Build history of the part. All positions in model axes, mm. A direction names the side the tool comes from. Coordinates: 2 decimals unless noted, no trailing zeros. Write each loop counter-clockwise with the first axis right and the second up, starting at its lowest first coordinate (ties: lowest second). Pieces come first, ordered by that corner, then holes. Notation, with made-up numbers: (-21.75, -18.75) -> (26.25, -18.75) arc R18 ccw to (26.25, 1.25) -> close; hole circle Ø7 at (58.25, 40). An arc over 180 degrees is marked (long way). Write each question's results on one line, items separated by ' | '. Start each with the question number.
Q1. Tool access for faces 5 (the face through (2, -8.75, 0)), 6 (the face through (5.4, -6.24, 0.01)), 7 (the face through (4, -3.75, 0)), 8 (the face through (-5.2, 6.5, 0)): list every direction of +Z, -Z, +X, -X, +Y, -Y with a clear straight run to the whole face (end or side of a thin tool).
Q2. Two-plate mould, pull along X, no slides. Class faces 1 (the face through (0, -2, 0.65)), 2 (the face through (-5.72, 7.67, 0.01)), 3 (the face through (5.8, -6, 0)), 4 (the face through (2.377, -7.359, 0.009)): released by +X, released by -X, zero draft, split by the parting line, or undercut.
Q3. Saw through at A-A on y = -5.25. Give the cut face in (x, z), and give its area (3 significant figures).
Q4. Saw through at C-C on x = -1.2. Give the cut face in (y, z).
Q5. Saw through at B-B on z = -0.45. Give the cut face in (x, y), and give its area (3 significant figures).
Q6. Drop flat-ended pins along their axis: pin 1 Ø0.6 at (x, z) = (4.5, 0) entering from +Y; pin 2 Ø0.6 at (y, z) = (0.5, 0) entering from -X. Give the stop position or say it passes through.
Q7. Drill centre lines: line 1 (Y direction, x = 2.25, z = 0.2); line 2 (Y direction, x = -3.5, z = 0.1); line 3 (X direction, y = -4.5, z = -0.6). Where is each one in solid material? Low to high.
Q8. Saw through at D-D on x = 4. Give the cut face in (y, z), and give its area (3 significant figures).
from build123d import *

# Parameters (mm, degrees)
SKETCH1_W           = 11.6
SKETCH1_H           = 17.5
BOSS_EXTRUDE1_DEPTH = 0.65
SKETCH2_R           = 1.25
SKETCH2_R_2         = 0.5
CUT_EXTRUDE1_DEPTH  = 11.577925127
SKETCH3_W           = 3.6
SKETCH3_H           = 14.7
CUT_EXTRUDE2_DEPTH  = 11.577925127
SKETCH4_W           = 0.6
SKETCH4_H           = 1
CUT_EXTRUDE3_DEPTH  = 11.577925127
FILLET2_R           = 0.2
CUT_EXTRUDE4_DEPTH  = 11.577925127
FILLET3_R           = 1
CHAMFER1_SIZE       = 0.2
FILLET4_R           = 0.5


with BuildPart() as part:
    # Sketch1 → Boss-Extrude1 (new, symmetric)
    with BuildSketch(Plane.XY):
        Rectangle(SKETCH1_W, SKETCH1_H)
    extrude(amount=BOSS_EXTRUDE1_DEPTH, both=True)

    # Sketch2 → Cut-Extrude1 (cut, through all)
    with BuildSketch(Plane.XY.offset(0.65)):
        with Locations((1.8, -6.25)):
            Circle(SKETCH2_R)
        with Locations((-1.2, -6.25)):
            Circle(SKETCH2_R_2)
        with BuildLine():
            Line((4.7, -5.75), (4.9, -5.75))
            ThreePointArc((4.9, -5.75), (5.4, -6.25), (4.9, -6.75))
            Line((4.9, -6.75), (4.7, -6.75))
            ThreePointArc((4.7, -6.75), (4.2, -6.25), (4.7, -5.75))
        make_face()
    extrude(amount=-CUT_EXTRUDE1_DEPTH, mode=Mode.SUBTRACT)

    # Sketch3 → Cut-Extrude2 (cut, through all)
    with BuildSketch(Plane.XY.offset(0.65)):
        with Locations((-4, -1.4)):
            Rectangle(SKETCH3_W, SKETCH3_H)
        Polygon((5.8, -3.75), (1.8, -3.75), (-0.8, 8.75), (5.8, 8.75), align=None)
    extrude(amount=-CUT_EXTRUDE2_DEPTH, mode=Mode.SUBTRACT)

    # Sketch4 → Cut-Extrude3 (cut, through all)
    with BuildSketch(Plane.XY.offset(0.65)):
        with Locations((-5.5, 6.45)):
            Rectangle(SKETCH4_W, SKETCH4_H)
    extrude(amount=-CUT_EXTRUDE3_DEPTH, mode=Mode.SUBTRACT)

    # Fillet2
    fillet2_edges = [part.edges().sort_by_distance(p)[0] for p in [
        (-5.2, 5.95, 0),
    ]]
    fillet(fillet2_edges, radius=FILLET2_R)

    # Sketch5 → Cut-Extrude4 (cut, through all)
    with BuildSketch(Plane.XY.offset(0.65)):
        Polygon((-5.8, 7.05), (-5.576190754, 8.75), (-5.8, 8.75), align=None)
    extrude(amount=-CUT_EXTRUDE4_DEPTH, mode=Mode.SUBTRACT)

    # Fillet3
    fillet3_edges = [part.edges().sort_by_distance(p)[0] for p in [
        (-2.2, 5.95, 0),
        (1.8, -3.75, 0),
        (-0.8, 8.75, 0),
    ]]
    fillet(fillet3_edges, radius=FILLET3_R)

    # Chamfer1
    chamfer1_edges = [part.edges().sort_by_distance(p)[0] for p in [
        (-2.2, -8.75, 0),
        (5.8, -3.75, 0),
        (5.8, -8.75, 0),
    ]]
    chamfer(chamfer1_edges, length=CHAMFER1_SIZE)

    # Fillet4
    fillet4_edges = [part.edges().sort_by_distance(p)[0] for p in [
        (-5.576190754, 8.75, 0),
    ]]
    fillet(fillet4_edges, radius=FILLET4_R)


solid = part.part
Returned:
1) face 5: +Z, -Z, +X, -X, -Y | face 6: +Z, -Z | face 7: +Z, -Z, +X, +Y | face 8: +Z, -Z, -X, -Y
2) face 1: zero draft | face 2: released by -X | face 3: released by +X | face 4: undercut
3) outline: (-2.2, -0.65) -> (1.05, -0.65) -> (1.05, 0.65) -> (-2.2, 0.65) -> close; (2.55, -0.65) -> (5.8, -0.65) -> (5.8, 0.65) -> (2.55, 0.65) -> close | area: 8.45 mm2
4) outline: (-8.75, -0.65) -> (-6.75, -0.65) -> (-6.75, 0.65) -> (-8.75, 0.65) -> close; (-5.75, -0.65) -> (8.66, -0.65) -> (8.66, 0.65) -> (-5.75, 0.65) -> close
5) outline: (-5.8, 6.95) -> (-5.2, 6.95) -> (-5.2, 6.15) arc R0.2 ccw to (-5, 5.95) -> (-3.2, 5.95) arc R1 cw to (-2.2, 4.95) -> (-2.2, -8.55) -> (-2, -8.75) -> (5.6, -8.75) -> (5.8, -8.55) -> (5.8, -3.95) -> (5.6, -3.75) -> (2.61, -3.75) arc R1 cw to (1.63, -2.95) -> (-0.63, 7.95) arc R1 ccw to (-1.61, 8.75) -> (-5.14, 8.75) arc R0.5 ccw to (-5.63, 8.32) -> (-5.8, 7.05) -> close; hole circle Ø1 at (-1.2, -6.25); hole circle Ø2.5 at (1.8, -6.25); hole (4.7, -6.75) -> (4.9, -6.75) arc R0.5 ccw to (4.9, -5.75) -> (4.7, -5.75) arc R0.5 ccw to start | area: 76.5 mm2
6) pin 1: stops at y = -3.75 | pin 2: stops at x = -2.2
7) line 1: y = -8.75 to -7.42, -5.08 to -3.68 | line 2: y = 5.95 to 8.75 | line 3: x = -2.2 to 5.8
8) outline: (-8.75, -0.65) -> (-3.75, -0.65) -> (-3.75, 0.65) -> (-8.75, 0.65) -> close | area: 6.50 mm2
